Input: dimensioned drawing with shaded views. Units: mm. Origin: part minimum x, y, z. A direction names the side the tool comes from. Coordinates: 2 decimals unless noted, no trailing zeros. Write each loop counter-clockwise with the first axis right and the second up, starting at its lowest first coordinate (ties: lowest second). Pieces come first, ordered by that corner, then holes. Notation, with made-up numbers: (30.25, 61) - (85.25, 61) arc R17 ccw to (85.25, 71) - close; hole circle Ø6 at (84, 5.25). An arc over 180 degrees is marked (long way). One line per question, with ' | ' between items.
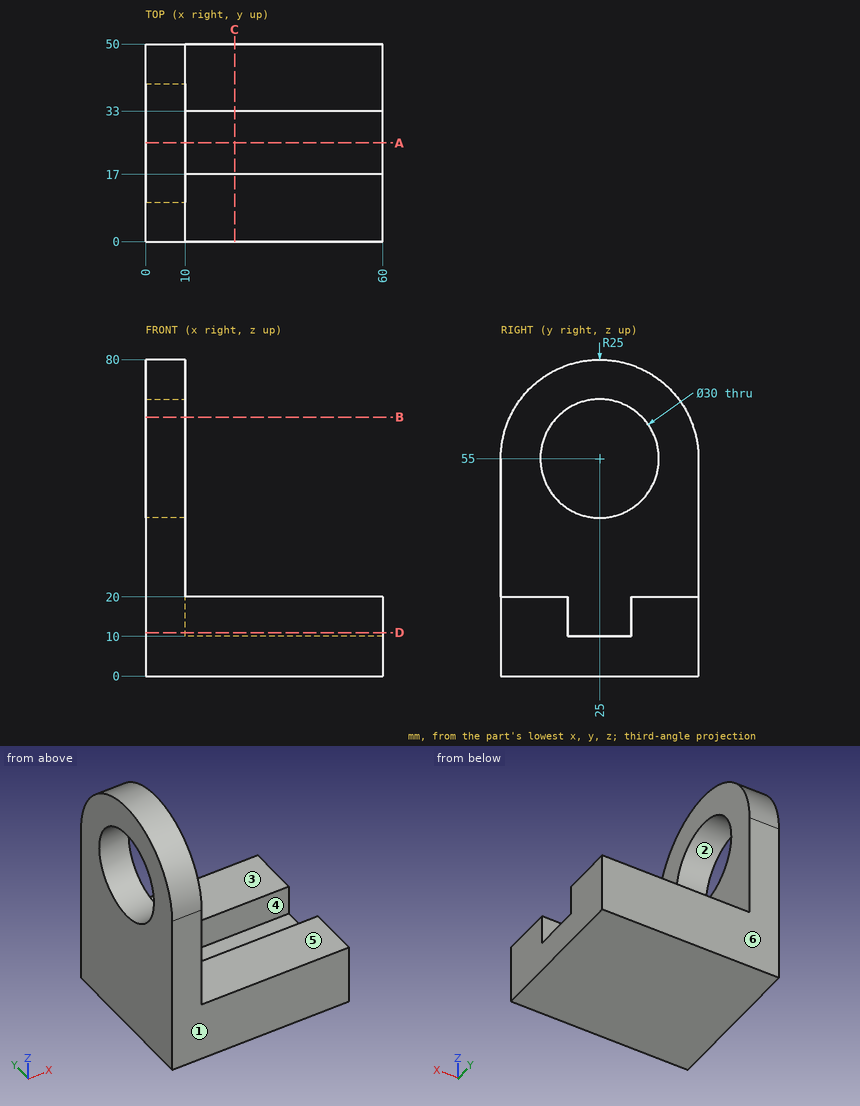
Item 1: Access query for the marked faces 4, 5 and 6. Directions: +Z, -Z, +X, -X, +Y, -Y. A direction counts if a zero-diameter tool reaches every point of the face in a straight line with its end or side. Return the directions, or none.
Check sheet entries:
face 4: +Z, +X | face 5: +Z, +X, +Y, -Y | face 6: +Z, -Z, +X, -X, +Y
Item 2: Cut plane A-A on y = 25. Return loops of the section in (x, z), and give its area (3 significant figures).
Check sheet entries:
outline: (0, 0) - (60, 0) - (60, 10) - (10, 10) - (10, 40) - (0, 40) - close; (0, 70) - (10, 70) - (10, 80) - (0, 80) - close | area: 1,000 mm²
Item 3: Cut plane B-B on z = 65.5. Return loops of the section in (x, y).
Check sheet entries:
outline: (0, 2.31) - (10, 2.31) - (10, 14.29) - (0, 14.29) - close; (0, 35.71) - (10, 35.71) - (10, 47.69) - (0, 47.69) - close
Item 4: Pin query (flat end, axial travel): pin 1 Ø13 at (x, y) = (31, 27.5) entering from +Z; pin 2 Ø15 at (y, z) = (12.5, 53) entering from +X. Return the tip coordinate at first contact, or that it passes through.
Check sheet entries:
pin 1: z = 20 | pin 2: x = 10
Item 5: Cut plane C-C on x = 22.5. Return loops of the section in (y, z).
Check sheet entries:
outline: (0, 0) - (50, 0) - (50, 20) - (33, 20) - (33, 10) - (17, 10) - (17, 20) - (0, 20) - close
Item 6: Ray query, line 1 along Y through (x, z) = (7.5, 55); line 2 along Y through (x, z) = (19, 11); line 3 along X through (y, z) = (47, 54). Return the intervals inside material, ascending. Write a range as [from, to].
Check sheet entries:
line 1: [0, 10], [40, 50] | line 2: [0, 17], [33, 50] | line 3: [0, 10]
Item 7: Mould query, pull axis Y, two halves, no side actions, for the marked faces 1, 2 and 3. Classes: pulls with the +Y half, pulls with the -Y half, needs draft (parallel to the pull), parting line crosses it, or undercut.
Check sheet entries:
face 1: pulls with the -Y half | face 2: undercut | face 3: needs draft
Item 8: Cut plane D-D on z = 11. Return loops of the section in (x, y), and give its area (3 significant figures).
Check sheet entries:
outline: (0, 0) - (60, 0) - (60, 17) - (10, 17) - (10, 33) - (60, 33) - (60, 50) - (0, 50) - close | area: 2,200 mm²
